Source: CAD feature listing. Evaluate the final solid. Frame: model axes, mm. Face numbers are marked on the shaded views. A direction names the side the tool comes from. Give positions to 0.01 mm unless a question says otherwise; leave off trailing zeros. Write each loop counter-clockwise with the first axis right and the second up, starting at its lowest first coordinate (ties: lowest second). Pieces come first, ordered by that corner, then holes. Notation, with made-up numbers: (50, -23.5) - (71, -23.5) arc R18 cw to (71, -7.5) - close; hole circle Ø11 at (-15, -9.75). An arc over 180 degrees is marked (long way). One line per question, with ' | ' between items. Start each with the question number.
(1) Section A-A, the plane y = 75.5. Return loops of the section in (x, z).
(2) Section C-C, the plane x = 47. Return loops of the section in (y, z), plus the area to 3 significant figures.
(3) Draft query along X for the marked faces 6, 7 and 8. Return one class per face: +X half, -X half, draft (parallel to the pull), parting line (faces both ways), or undercut.
(4) Ray query, line 1 (X direction, y = 12, z = 155); line 2 (Y direction, x = -32, z = 101); line 3 (Y direction, x = 8.5, z = 152). Return the intervals inside material, ascending. Write a range as [from, to].
(5) Pin query (flat end, axial travel): pin 1 (11 mm diameter, centred on x = 78.5, z = 55.5, fed in from +Y); pin 2 (5 mm diameter, centred on y = 49.5, z = 35.5, fed in from -X); pin 3 (9.5 mm diameter, centred on x = 28, z = 53.5, fed in from +Y). Return the tip coordinate at first contact, or that it passes through.
(6) Section D-D, the plane z = 140. Return loops of the section in (x, y).
(7) Section B-B, the plane x = 28.5. Return loops of the section in (y, z), plus the area to 3 significant figures.
(8) Access query for the marked faces 1, 2, 3, 4 and 5. Directions: +Z, -Z, +X, -X, +Y, -Y. A direction counts if a zero-diameter tool reaches every point of the face in a straight line with its end or side. Return the directions, or none.
```python
from build123d import *

# Parameters (mm, degrees)
V_BLOCK_BODY_DEPTH     = 125
MOUNTING_LUGS_SKETCH_R = 10.5
MOUNTING_LUGS_DEPTH    = 20


with BuildPart() as part:
    # V-Block Profile Sketch → V-Block Body (new body)
    with BuildSketch(Plane.XY):
        Polygon((-40.458015267, 0), (84.541984733, 0), (84.541984733, 36), (74.541984733, 36), (74.541984733, 56), (84.541984733, 56), (84.541984733, 96), (72.041984733, 96), (31.052534351, 52), (31.052534351, 46), (19.052534351, 46), (19.052534351, 52.989450382), (-27.958015267, 100), (-40.458015267, 100), (-40.458015267, 56), (-30.458015267, 56), (-30.458015267, 36), (-40.458015267, 36), align=None)
    extrude(amount=V_BLOCK_BODY_DEPTH)

    # Mounting Lugs Sketch → Mounting Lugs (add)
    with BuildSketch(Plane.XZ):
        with BuildLine():
            Line((52.421361688, 155), (52.421361688, -30))
            ThreePointArc((52.421361688, -30), (22.421361688, -60), (-7.578638312, -30))
            Line((-7.578638312, -30), (-7.578638312, 155))
            ThreePointArc((-7.578638312, 155), (22.421361688, 185), (52.421361688, 155))
        make_face()
        with Locations(Location((22.421361688, 155, 0), (0, 0, 270))):
            Circle(MOUNTING_LUGS_SKETCH_R, mode=Mode.SUBTRACT)
        with Locations(Location((22.421361688, -30, 0), (0, 0, 270))):
            Circle(MOUNTING_LUGS_SKETCH_R, mode=Mode.SUBTRACT)
    extrude(amount=-MOUNTING_LUGS_DEPTH)


solid = part.part
```
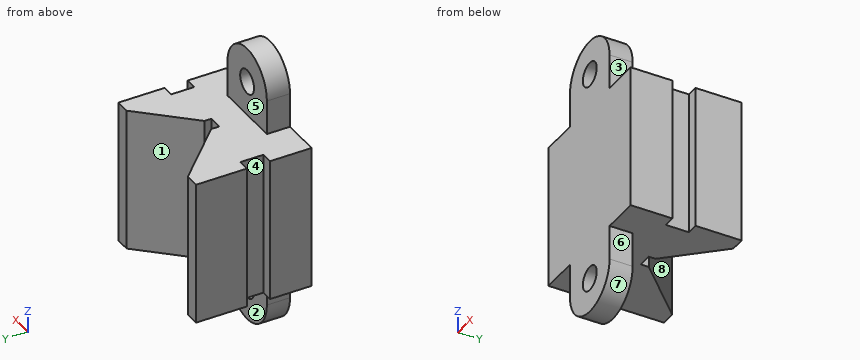
Check sheet entries:
1) outline: (-40.46, 0) - (-3.46, 0) - (-3.46, 125) - (-40.46, 125) - close; (52.94, 0) - (84.54, 0) - (84.54, 125) - (52.94, 125) - close
2) outline: (0, -47.2) - (20, -47.2) - (20, 0) - (69.12, 0) - (69.12, 125) - (20, 125) - (20, 172.2) - (0, 172.2) - close | area: 10,500 mm²
3) face 6: +X half | face 7: parting line | face 8: undercut
4) line 1: [-7.58, 11.92], [32.92, 52.42] | line 2: [0, 36], [56, 100] | line 3: [0, 20]
5) pin 1: y = 96 | pin 2: x = -30.46 | pin 3: y = 53.82
6) outline: (-7.58, 0) - (52.42, 0) - (52.42, 20) - (-7.58, 20) - close
7) outline: (0, -59.38) - (20, -59.38) - (20, -38.56) - (0, -38.56) - close; (0, -21.44) - (20, -21.44) - (20, 0) - (46, 0) - (46, 125) - (20, 125) - (20, 146.44) - (0, 146.44) - close; (0, 163.56) - (20, 163.56) - (20, 184.38) - (0, 184.38) - close | area: 7,440 mm²
8) face 1: +Z, -Z, +Y | face 2: -Z, +X, -X, +Y | face 3: +Z, +X, +Y, -Y | face 4: +Z, -Z, -X | face 5: +Z, +X, -X, +Y
